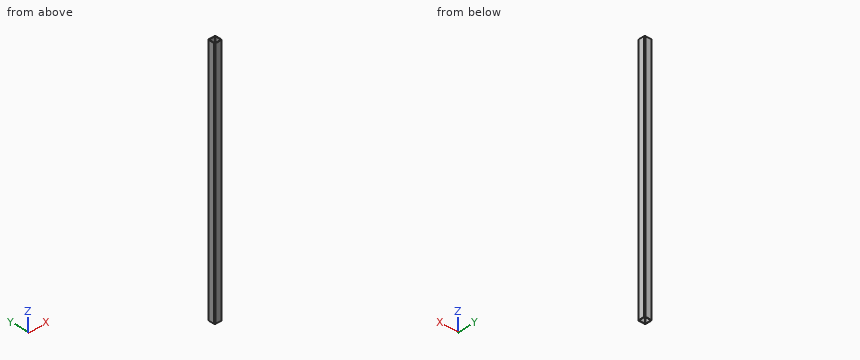
```python
from build123d import *

# Parameters (mm, degrees)
EXTRUDE_THIN1_DEPTH = 518.8


with BuildPart() as part:
    # Sketch1 → Extrude-Thin1 (new, symmetric)
    with BuildSketch(Plane.XY):
        with BuildLine():
            Line((-15, 11), (-15, -11))
            ThreePointArc((-15, -11), (-13.828427125, -13.828427125), (-11, -15))
            Line((-11, -15), (11, -15))
            ThreePointArc((11, -15), (13.828427125, -13.828427125), (15, -11))
            Line((15, -11), (15, 11))
            ThreePointArc((15, 11), (13.828427125, 13.828427125), (11, 15))
            Line((11, 15), (-11, 15))
            ThreePointArc((-11, 15), (-13.828427125, 13.828427125), (-15, 11))
        make_face()
        with BuildLine():
            Line((-13, 11), (-13, -11))
            ThreePointArc((-13, -11), (-12.414213562, -12.414213562), (-11, -13))
            Line((-11, -13), (11, -13))
            ThreePointArc((11, -13), (12.414213562, -12.414213562), (13, -11))
            Line((13, -11), (13, 11))
            ThreePointArc((13, 11), (12.414213562, 12.414213562), (11, 13))
            Line((11, 13), (-11, 13))
            ThreePointArc((-11, 13), (-12.414213562, 12.414213562), (-13, 11))
        make_face(mode=Mode.SUBTRACT)
    extrude(amount=EXTRUDE_THIN1_DEPTH, both=True)


solid = part.part
```
Can you work these out from the model? Positions are in its coordinate system, mm. Give positions to 0.01 mm unless a question says otherwise; leave off trailing zeros. Write each loop counter-clockwise with the first axis right and the second up, starting at its lowest first coordinate (ties: lowest second). Pieces come first, ordered by that corner, then holes. Notation, with made-up numbers: (-9, -17.75) - (49, -17.75) arc R17 ccw to (49, -13.75) - close; hole circle Ø1 at (68, 3.5). An arc over 180 degrees is marked (long way). Write item = value, one per line. Start each with the question number.
1. Imagine slicing it at B-B (y = 2). Please give me the cut outline in (x, z).
2. Imagine slicing it at A-A (z = -422.5). Please give me the cut outline in (x, y), and give its area (3 significant figures).
3. Please list where these lines run through material, in increasing order: line 1 (Y direction, x = -3.5, z = 143); line 2 (X direction, y = 13.5, z = -298).
4. For pin 1 (2 mm diameter, centred on y = 12, z = 188.5, fed in from +X), with a flat end and sliding along its axis, tell me the tip position at first contact or that it passes through.
Worked answers:
q1.outline = (-15, -518.8) - (-13, -518.8) - (-13, 518.8) - (-15, 518.8) - close; (13, -518.8) - (15, -518.8) - (15, 518.8) - (13, 518.8) - close
q2.outline = (-15, -11) arc R4 ccw to (-11, -15) - (11, -15) arc R4 ccw to (15, -11) - (15, 11) arc R4 ccw to (11, 15) - (-11, 15) arc R4 ccw to (-15, 11) - close; hole (-13, -11) arc R2 ccw to (-11, -13) - (11, -13) arc R2 ccw to (13, -11) - (13, 11) arc R2 ccw to (11, 13) - (-11, 13) arc R2 ccw to (-13, 11) - close
q2.area = 214 mm2
q3.line_1 = -15 to -13, 13 to 15
q3.line_2 = -14.12 to 14.12
q4.pin_1 = 15
